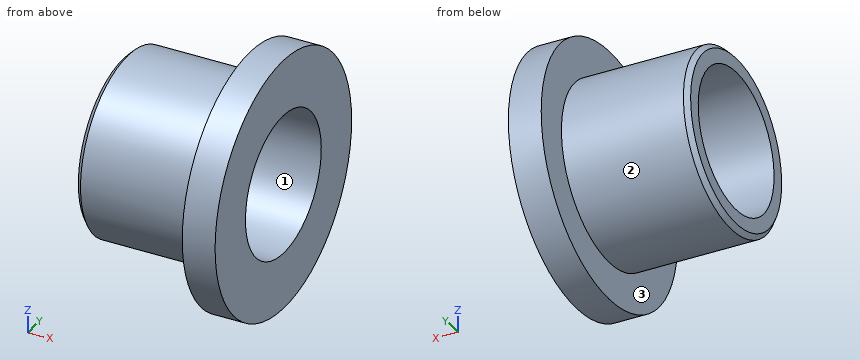
```python
from build123d import *

# Parameters (mm, degrees)
CHAMFER1_SIZE = 1


with BuildPart() as part:
    # Sketch1 → Revolve1 (revolve)
    with BuildSketch(Plane.XY, mode=Mode.PRIVATE) as revolve1_sk:
        Polygon((0, 15), (34, 15), (34, 27), (27, 27), (27, 19), (0, 19), align=None)
    revolve(revolve1_sk.sketch.rotate(Axis((0, 0, 0), (1, 0, 0)), 90), axis=Axis((0, 0, 0), (1, 0, 0)))

    # Chamfer1
    chamfer1_edges = [part.edges().sort_by_distance(p)[0] for p in [
        (0, 0, -19),
    ]]
    chamfer(chamfer1_edges, length=CHAMFER1_SIZE)


solid = part.part
```
For this review, take the finished solid that the model builds, in its own axes (mm). Face numbers are marked on the shaded views. Coordinates: 2 decimals unless noted, no trailing zeros. Write each loop counter-clockwise with the first axis right and the second up, starting at its lowest first coordinate (ties: lowest second). Pieces come first, ordered by that corner, then holes.
(1) The part is to be moulded in two halves that separate along Y. For the marked faces 1, 2 and 3, say which applies: +Y half, -Y half, draft (parallel to the pull), parting line (faces both ways), or undercut.
(2) Wall thickness on probe 1 along Y at (x, z) = (23, 0); probe 2 along X at (y, z) = (22, 0); probe 3 along Z at (x, y) = (18, -3.5): over which ranges is each line inside the solid? List them lowest first.
(3) Add section C-C on x = 14.5. Give the boundary of the cut face in (y, z), then the cut area to 3 significant figures.
(4) Add section D-D on y = 21. Give the boundary of the cut face in (x, z).
(5) Add section A-A on y = 0. Give the boundary of the cut face in (x, z).
(6) For pin 1 Ø12 at (y, z) = (-8.5, -1.5) entering from -X; pin 2 Ø8 at (x, z) = (6, 6.5) entering from -Y; pin 3 Ø8 at (x, z) = (25, 9) entering from +Y; pin 4 Ø3 at (x, y) = (17, -18) entering from -Z, all flat-tipped, find the tip position at first contact; note any pin that passes through.
Answer sheet:
1. face 1: undercut
1. face 2: parting line
1. face 3: draft
2. probe 1: y = -19 to -15, 15 to 19
2. probe 2: x = 27 to 34
2. probe 3: z = -18.67 to -14.59, 14.59 to 18.67
3. outline: circle Ø38 at (0, 0); hole circle Ø30 at (0, 0)
3. area: 427 mm2
4. outline: (27, -16.97) - (34, -16.97) - (34, 16.97) - (27, 16.97) - close
5. outline: (0, -18) - (1, -19) - (27, -19) - (27, -27) - (34, -27) - (34, -15) - (0, -15) - close; (0, 15) - (34, 15) - (34, 27) - (27, 27) - (27, 19) - (1, 19) - (0, 18) - close
6. pin 1: passes through
6. pin 2: stops at y = -18.83
6. pin 3: stops at y = 26.43
6. pin 4: stops at z = -9.42
